Could you check a few things on this model? Use its own coordinates, in mm. A direction names the side the tool comes from. Coordinates: 2 decimals unless noted, no trailing zeros. Loops run counter-clockwise (first coordinate to the right, second up) from the corner with the lowest first, then second, coordinate; pieces in that order, holes last.
from build123d import *

# Parameters (mm, degrees)
SKETCH1_R           = 75
SKETCH1_R_2         = 50
BOSS_EXTRUDE1_DEPTH = 120
SKETCH2_W           = 38.391183042
SKETCH2_H           = 72.968672404
CUT_EXTRUDE1_DEPTH  = 161.15617378
CIRPATTERN1_COUNT   = 4


with BuildPart() as part:
    # Sketch1 → Boss-Extrude1 (new body)
    with BuildSketch(Plane.XY):
        Circle(SKETCH1_R)
        Circle(SKETCH1_R_2, mode=Mode.SUBTRACT)
    extrude(amount=BOSS_EXTRUDE1_DEPTH)

    # Sketch2 → Cut-Extrude1 (cut, through all)
    with BuildSketch(Plane(origin=(0, 0, 0), x_dir=(1, 0, 0), z_dir=(0, 1, 0))):
        with Locations((0, -60)):
            Rectangle(SKETCH2_W, SKETCH2_H)
    cut_extrude1 = extrude(amount=-CUT_EXTRUDE1_DEPTH, mode=Mode.SUBTRACT)

    # CirPattern1: Cut-Extrude1 ×4 about axis
    cirpattern1_axis = Axis((0, 0, 0), (0, 0, 1))
    for i in range(1, CIRPATTERN1_COUNT):
        add(cut_extrude1.rotate(cirpattern1_axis, i * 360 / CIRPATTERN1_COUNT), mode=Mode.SUBTRACT)


solid = part.part
(1) Imagine slicing it at A-A, the plane z = 52.5. Write out the boundary of the cut face in (x, y).
Answers:
outline: (-72.5, -19.2) arc R75 ccw to (-19.2, -72.5) - (-19.2, -46.17) arc R50 cw to (-46.17, -19.2) - close; (-72.5, 19.2) - (-46.17, 19.2) arc R50 cw to (-19.2, 46.17) - (-19.2, 72.5) arc R75 ccw to start; (19.2, -72.5) arc R75 ccw to (72.5, -19.2) - (46.17, -19.2) arc R50 cw to (19.2, -46.17) - close; (19.2, 46.17) arc R50 cw to (46.17, 19.2) - (72.5, 19.2) arc R75 ccw to (19.2, 72.5) - close
(2) For pin 1 (5 mm diameter, centred on y = -8, z = 93, fed in from +X); pin 2 (5 mm diameter, centred on x = 58, z = 73.5, fed in from -Y); pin 3 (13 mm diameter, centred on x = -64.5, z = 49, fed in from +Y); pin 4 (8 mm diameter, centred on x = -64, z = 58, fed in from -Y), each with a flat end and sliding along its axis, tell me the tip position at first contact or that it passes through.
Answers:
pin 1: passes through
pin 2: stops at y = -50.45
pin 3: stops at y = 47.55
pin 4: stops at y = -45
(3) Which directions (+Z, -Z, +X, -X, +Y, -Y) give clear straight access to the entire face, cutting with the end or side of a thin tool? Please do faces 5 (the face through (-59, 19.196, 61)), 6 (the face through (0, -60, 96.484)), 7 (the face through (49, -16, 0)).
Answers:
face 5: +X, -X
face 6: +Y, -Y
face 7: -Z, +X, -X, +Y, -Y
(4) Imagine slicing it at D-D, the plane x = -40.5. Write out the boundary of the cut face in (y, z).
Answers:
outline: (-63.12, 0) - (-29.32, 0) - (-29.32, 120) - (-63.12, 120) - close; (29.32, 0) - (63.12, 0) - (63.12, 120) - (29.32, 120) - close
(5) We'd pull the mould along Y, two halves only. Please class faces 1 (the face through (-40, -30, 59)), 2 (the face through (71.537, 22.528, 59.16)), 3 (the face through (19.196, -59, 61)), 4 (the face through (-59, -19.196, 61)): +Y half, -Y half, draft (parallel to the pull), parting line (faces both ways), or undercut.
Answers:
face 1: undercut
face 2: parting line
face 3: draft
face 4: undercut
(6) Imagine slicing it at C-C, the plane y = 24. Write out the boundary of the cut face in (x, z), and give its area (3 significant figures).
Answers:
outline: (-71.06, 0) - (-43.86, 0) - (-43.86, 120) - (-71.06, 120) - close; (43.86, 0) - (71.06, 0) - (71.06, 120) - (43.86, 120) - close
area: 6,530 mm2
(7) Imagine slicing it at B-B, the plane x = 0. Write out the boundary of the cut face in (y, z).
Answers:
outline: (-75, 0) - (-50, 0) - (-50, 23.52) - (-75, 23.52) - close; (-75, 96.48) - (-50, 96.48) - (-50, 120) - (-75, 120) - close; (50, 0) - (75, 0) - (75, 23.52) - (50, 23.52) - close; (50, 96.48) - (75, 96.48) - (75, 120) - (50, 120) - close
(8) I need wall thicknesses on probe 1 along Z at (x, y) = (-65.5, -18); probe 2 along Y at (x, z) = (-51.5, 61.5); probe 3 along X at (y, z) = (-57, 34). Which ranges of each line are inside material? Lowest first, please.
Answers:
probe 1: z = 0 to 23.52, 96.48 to 120
probe 2: y = -54.52 to -19.2, 19.2 to 54.52
probe 3: x = -48.74 to -19.2, 19.2 to 48.74
